from build123d import *

# Parameters (mm, degrees)
FLANGE_SKETCH_R             = 45
FLANGE_SKETCH_R_2           = 15
FLANGE_90_DEPTH             = 14.2
HUB_SKETCH_R                = 20
HUB_SKETCH_R_2              = 15
HUB_40_DEPTH                = 44.2
COLLAR_SKETCH_R             = 25
COLLAR_SKETCH_R_2           = 15
COLLAR_50_DEPTH             = 6
END_SLEEVE_SKETCH_R         = 25
END_SLEEVE_SKETCH_R_2       = 19
END_SLEEVE_50_BORE_38_DEPTH = 24
FLANGE_EDGE_CHAMFER_SIZE    = 3
FLANGE_EDGE_CHAMFER_SIZE2   = 3.5
BOLT_HOLES_SET_A_SKETCH_R   = 6.25
BOLT_HOLES_SET_A_DEPTH      = 24
BOLT_HOLES_SET_B_SKETCH_R   = 6.25
BOLT_HOLES_SET_B_DEPTH      = 24


with BuildPart() as part:
    # Flange Sketch → Flange Ø90 (new body)
    with BuildSketch(Plane.XY):
        Circle(FLANGE_SKETCH_R)
        Circle(FLANGE_SKETCH_R_2, mode=Mode.SUBTRACT)
    extrude(amount=FLANGE_90_DEPTH)

    # Hub Sketch → Hub Ø40 (add)
    with BuildSketch(Plane.XY.offset(14.2)):
        Circle(HUB_SKETCH_R)
        Circle(HUB_SKETCH_R_2, mode=Mode.SUBTRACT)
    extrude(amount=HUB_40_DEPTH)

    # Collar Sketch → Collar Ø50 (add)
    with BuildSketch(Plane.XY.offset(58.4)):
        Circle(COLLAR_SKETCH_R)
        Circle(COLLAR_SKETCH_R_2, mode=Mode.SUBTRACT)
    extrude(amount=COLLAR_50_DEPTH)

    # End Sleeve Sketch → End Sleeve Ø50 Bore Ø38 (add)
    with BuildSketch(Plane.XY.offset(64.4)):
        Circle(END_SLEEVE_SKETCH_R)
        Circle(END_SLEEVE_SKETCH_R_2, mode=Mode.SUBTRACT)
    extrude(amount=END_SLEEVE_50_BORE_38_DEPTH)

    # Flange Edge Chamfer
    flange_edge_chamfer_edges = [part.edges().sort_by_distance(p)[0] for p in [
        (-15, 0, 0),
    ]]
    flange_edge_chamfer_side = [part.faces().sort_by_distance(p)[0] for p in [
        (-15, 0, 32.2),
    ]]
    chamfer(flange_edge_chamfer_edges, length=FLANGE_EDGE_CHAMFER_SIZE, length2=FLANGE_EDGE_CHAMFER_SIZE2, reference=flange_edge_chamfer_side[0])

    # Bolt Holes Set A Sketch → Bolt Holes Set A (cut)
    with BuildSketch(Plane.XY):
        with Locations((0, 32.5)):
            Circle(BOLT_HOLES_SET_A_SKETCH_R)
        with Locations((0, -32.5)):
            Circle(BOLT_HOLES_SET_A_SKETCH_R)
    extrude(amount=BOLT_HOLES_SET_A_DEPTH, mode=Mode.SUBTRACT)

    # Bolt Holes Set B Sketch → Bolt Holes Set B (cut)
    with BuildSketch(Plane.XY):
        with Locations((-32.5, 0)):
            Circle(BOLT_HOLES_SET_B_SKETCH_R)
        with Locations((32.5, 0)):
            Circle(BOLT_HOLES_SET_B_SKETCH_R)
    extrude(amount=BOLT_HOLES_SET_B_DEPTH, mode=Mode.SUBTRACT)


solid = part.part
Here's how the part is built. I have some questions about the finished solid (model axes, mm). A direction names the side the tool comes from. Give positions to 0.01 mm unless a question says otherwise; leave off trailing zeros. Order: outer loops, then holes, each group sorted by start corner. A loop starts at its lowest first (then second) coordinate and runs counter-clockwise, first axis right, second up. Notation, with made-up numbers: M 87,-16 L 119,-16 A25 cw 119,5 Z; hole C 11,12 d10. An arc over 180 degrees is marked long. Answer as a JSON object with one key per item and string values. Group by question number.
1) Suppose I cut it at A-A, the plane x = 0. Count the separate pieces of the cut face and the enclosed holes in it, plus the area to 3 significant figures.
2) Suppose I cut it at D-D, the plane x = 36. Write out the boundary of the cut face in (y, z), plus the area to 3 significant figures.
3) On a 3-axis mill with a long thin cutter (end or side, diameter ignored), from which of +Z, -Z, +X, -X, +Y, -Y can I reach the whole of each face in a straight line? I mean faces 1 (the flat face through (14, 6, 64.4)), 2 (the cylindrical face through (-4.336, -19.524, 35.991)), 3 (the conical face through (7.023, -13.502, 2.812)). Say none if no direction works.
4) We'd pull the mould along X, two halves only. Please class faces 4 (the flat face through (-11, 17, 58.4)), 5 (the cylindrical face through (20.765, -39.923, 7.001)), 6 (the cylindrical face through (-14.985, 0.66, 33.27)), 7 (the cylindrical face through (-0.8, 38.7, 7)): pulls with the +X half, pulls with the -X half, needs draft (parallel to the pull), parting line crosses it, or undercut.
5) Please list where these lines run through material, in increasing order: L1, parallel to Y at x = 0, z = 75; L2, parallel to Y at x = 0, z = 10; L3, parallel to Z at x = 17, y = -13.5. Write a range as [from, to].
6) I'm going to push flat-ended pins straight in: pin 1 Ø1.5 at (x, y) = (-24.5, -15.5) entering from +Z; pin 2 Ø6 at (x, z) = (11.5, 35.5) entering from +Y; pin 3 Ø14.5 at (x, y) = (-32.5, 0) entering from -Z; pin 4 Ø12 at (x, y) = (2.5, -12) entering from -Z. Where does each tip first touch, or does it pass through?
7) Suppose I cut it at C-C, the plane z = 8. Write out the boundary of the cut face in (x, y), plus the area to 3 significant figures.
8) Suppose I cut it at B-B, the plane y = -28.5. Write out the boundary of the cut face in (x, z), plus the area to 3 significant figures.
Results found:
{
 "1": {"separate pieces": "4", "enclosed holes": "0", "area": "1,340 mm²"},
 "2": {"outline": "M -27,0 L -5.18,0 L -5.18,14.2 L -27,14.2 Z; M 5.18,0 L 27,0 L 27,14.2 L 5.18,14.2 Z", "area": "620 mm²"},
 "3": {"face 1": "+Z", "face 2": "none", "face 3": "-Z"},
 "4": {"face 4": "needs draft", "face 5": "parting line crosses it", "face 6": "undercut", "face 7": "undercut"},
 "5": {"L1": "[-25, -19], [19, 25]", "L2": "[-45, -38.75], [-26.25, -15], [15, 26.25], [38.75, 45]", "L3": "[0, 14.2], [58.4, 88.4]"},
 "6": {"pin 1": "z = 14.2", "pin 2": "y = 18.1", "pin 3": "z = 0", "pin 4": "z = 0.21"},
 "7": {"outline": "C 0,0 d90; hole C -32.5,0 d12.5; hole C 0,0 d30; hole C 0,-32.5 d12.5; hole C 0,32.5 d12.5; hole C 32.5,0 d12.5", "area": "5,160 mm²"},
 "8": {"outline": "M -34.82,0 L -4.8,0 L -4.8,14.2 L -34.82,14.2 Z; M 4.8,0 L 34.82,0 L 34.82,14.2 L 4.8,14.2 Z", "area": "853 mm²"}
}
